Work out the finished part from the listing and answer in its coordinate system (mm). A direction names the side the tool comes from. Coordinates: 2 decimals unless noted, no trailing zeros. Loops run counter-clockwise (first coordinate to the right, second up) from the corner with the lowest first, then second, coordinate; pieces in that order, holes last. Notation, with made-up numbers: (-31.5, 57.5) -> (22.5, 57.5) arc R14 cw to (22.5, 61.5) -> close; hole circle Ø3 at (-31, -5). An arc over 180 degrees is marked (long way). Use a Markdown table: item, result. Add a question column.
```python
from build123d import *

# Parameters (mm, degrees)
FILLET1_R = 0.3
FILLET2_R = 0.3


with BuildPart() as part:
    # Sketch1 → Revolve1 (revolve)
    with BuildSketch(Plane.XY, mode=Mode.PRIVATE) as revolve1_sk:
        Polygon((0, 25), (7, 25), (7, 26.45), (6.68, 26.45), (6.68, 31), (7, 31), (7, 32.5), (0, 32.5), (0, 31), (0.32, 31), (0.32, 26.45), (0, 26.45), align=None)
    revolve(revolve1_sk.sketch.rotate(Axis((0, 0, 0), (1, 0, 0)), 90), axis=Axis((0, 0, 0), (1, 0, 0)))

    # Fillet1
    fillet1_edges = [part.edges().sort_by_distance(p)[0] for p in [
        (0, 0, -32.5),
        (7, 0, -32.5),
    ]]
    fillet(fillet1_edges, radius=FILLET1_R)

    # Fillet2
    fillet2_edges = [part.edges().sort_by_distance(p)[0] for p in [
        (7, 0, -25),
        (0, 0, -25),
    ]]
    fillet(fillet2_edges, radius=FILLET2_R)


solid = part.part
```
Item 1: Section C-C (x = 3) is taken. Determine the outline of the cut face in (y, z), then the cut area to 3 significant figures.
Item 2: Given pin 1 (2 mm diameter, centred on x = 5.5, z = 22, fed in from +Y); pin 2 (4 mm diameter, centred on x = 1, y = 4.5, fed in from +Z); pin 3 (1.5 mm diameter, centred on x = 3, z = -3.5, fed in from -Y), each flat-ended and moving along its own axis, determine where each tip first touches the part or whether it passes through.
Item 3: For faces 4 (the face through (3.545, -7.509, 23.846)), 5 (the face through (6.838, 16.094, -20.99)), 6 (the face through (0.158, 16.094, -20.99)), determine the directions among +Z, -Z, +X, -X, +Y, -Y from which every point of the face is accessible in a straight line to the end or side of a thin tool.
Item 4: For a pull along Z with two mould halves and no side action, classify faces 1 (the face through (6.68, -14, -23)), 2 (the face through (3.46, -9.76, 31)), 3 (the face through (0, -26.4, -16.8)) as +Z half, -Z half, draft (parallel to the pull), parting line (faces both ways), or undercut.
Item 5: Find the intervals of material crossed by probe 1 along Y at (x, z) = (4.75, 0); probe 2 along Z at (x, y) = (6.75, -9.5); probe 3 along Y at (x, z) = (0.2, 0), in increasing order.
Output:
| question | item | result |
|---|---|---|
| 1 | outline | circle Ø65 at (0, 0); hole circle Ø50 at (0, 0) |
| 1 | area | 1,350 mm2 |
| 2 | pin 1 | stops at y = 24.8 |
| 2 | pin 2 | stops at z = 32.4 |
| 2 | pin 3 | stops at y = -32.38 |
| 3 | face 4 | +X, -X |
| 3 | face 5 | +X |
| 3 | face 6 | -X |
| 4 | face 1 | undercut |
| 4 | face 2 | parting line |
| 4 | face 3 | draft |
| 5 | probe 1 | y = -32.5 to -25, 25 to 32.5 |
| 5 | probe 2 | z = -31.08 to -29.51, -24.69 to -23.13, 23.13 to 24.69, 29.51 to 31.08 |
| 5 | probe 3 | y = -32.48 to -31, -26.45 to -25.02, 25.02 to 26.45, 31 to 32.48 |
